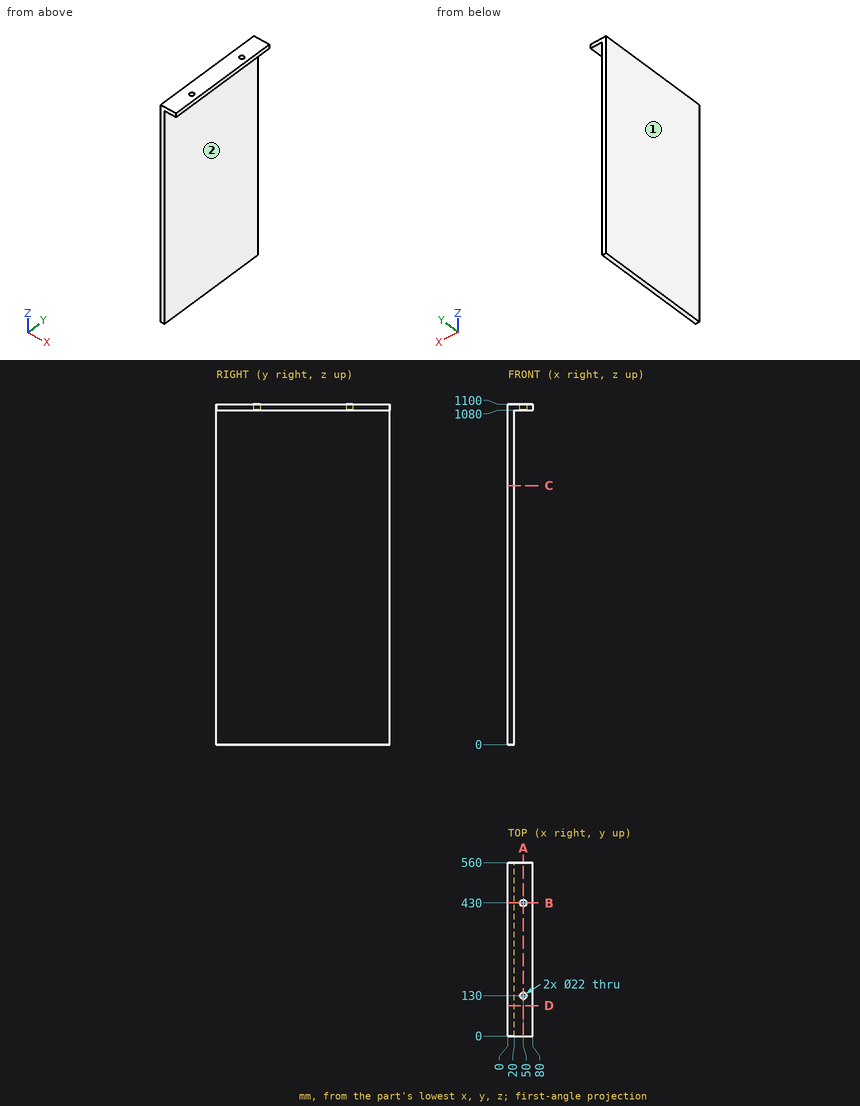
Geometry check sheet. Reference: drawing and pictorial views, mm from the part's lowest x, y, z. A direction names the side the tool comes from. Coordinates: 2 decimals unless noted, no trailing zeros. Order: outer loops, then holes, each group sorted by start corner. A loop starts at its lowest first (then second) coordinate and runs counter-clockwise, first axis right, second up.
Item 1: Material ranges on L1, parallel to Y at x = 50, z = 1084.5; L2, parallel to X at y = 410, z = 338.5; L3, parallel to Z at x = 54, y = 304, recorded low to high.
Filled in:
L1: y = 0 to 119, 141 to 419, 441 to 560
L2: x = 0 to 20
L3: z = 1080 to 1100
Item 2: Section check C-C, the plane z = 836. Enter the section's corners in (x, y), then the cut area to 3 significant figures.
Filled in:
outline: (0, 0) - (20, 0) - (20, 560) - (0, 560) - close
area: 11,200 mm2
Item 3: Access from +Z, -Z, +X, -X, +Y, -Y to the whole of each face (thin tool, end or side, straight path). Record for the marked faces 1 and 2.
Filled in:
face 1: +Z, -Z, -X, +Y, -Y
face 2: -Z, +X, +Y, -Y
Item 4: Section check D-D, the plane y = 98.5. Enter the section's corners in (x, z).
Filled in:
outline: (0, 0) - (20, 0) - (20, 1080) - (80, 1080) - (80, 1100) - (0, 1100) - close
Item 5: Depth check by flat-ended pin: pin 1 (18 mm diameter, centred on x = 58.5, y = 349.5, fed in from -Z); pin 2 (8 mm diameter, centred on y = 133, z = 201.5, fed in from +X). Enter the tip coordinate at first touch or a pass-through.
Filled in:
pin 1: stops at z = 1080
pin 2: stops at x = 20
Item 6: Section check A-A, the plane x = 50. Enter the section's corners in (y, z), then the cut area to 3 significant figures.
Filled in:
outline: (0, 1080) - (119, 1080) - (119, 1100) - (0, 1100) - close; (141, 1080) - (419, 1080) - (419, 1100) - (141, 1100) - close; (441, 1080) - (560, 1080) - (560, 1100) - (441, 1100) - close
area: 10,300 mm2
Item 7: Section check B-B, the plane y = 430. Enter the section's corners in (x, z).
Filled in:
outline: (0, 0) - (20, 0) - (20, 1080) - (39, 1080) - (39, 1100) - (0, 1100) - close; (61, 1080) - (80, 1080) - (80, 1100) - (61, 1100) - close
